Input: part model. Units: mm. Frame: model coordinates. Face numbers are marked on the shaded views. Coordinates: 2 decimals unless noted, no trailing zeros. Loops run counter-clockwise (first coordinate to the right, second up) from the corner with the lowest first, then second, coordinate; pieces in that order, holes last.
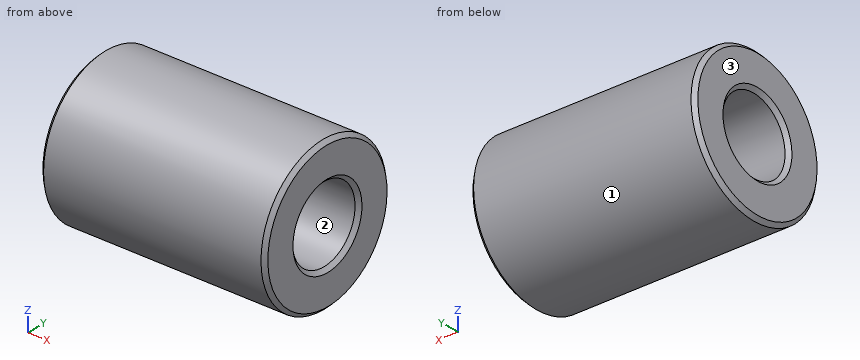
```python
from build123d import *

# Parameters (mm, degrees)
CHAMFER1_SIZE = 0.2


with BuildPart() as part:
    # Sketch1 → Revolve1 (revolve)
    with BuildSketch(Plane.XY, mode=Mode.PRIVATE) as revolve1_sk:
        Polygon((0, 3.7), (0, 2), (12, 2), (12, 3.7), (12, 4), (11.7, 4), (0.3, 4), (0, 4), align=None)
    revolve(revolve1_sk.sketch.rotate(Axis((12, 0, 0), (-1, 0, 0)), 270), axis=Axis((12, 0, 0), (-1, 0, 0)))

    # Chamfer1
    chamfer1_edges = [part.edges().sort_by_distance(p)[0] for p in [
        (0, 0, -4),
        (12, 0, -4),
        (12, 0, -2),
        (0, 0, -2),
    ]]
    chamfer(chamfer1_edges, length=CHAMFER1_SIZE)


solid = part.part
```
Item 1: Section query A-A (z = 0). Output: boundary loops of the cut face in (x, y).
Result:
outline: (0, -3.8) - (0.2, -4) - (11.8, -4) - (12, -3.8) - (12, -2.2) - (11.8, -2) - (0.2, -2) - (0, -2.2) - close; (0, 2.2) - (0.2, 2) - (11.8, 2) - (12, 2.2) - (12, 3.8) - (11.8, 4) - (0.2, 4) - (0, 3.8) - close
Item 2: Line query: L1, parallel to Y at x = 7.5, z = 0; L2, parallel to Z at x = 5, y = -1; L3, parallel to Z at x = 3.75, y = 1.25. Output: solid intervals per line, ascending.
Result:
L1: y = -4 to -2, 2 to 4
L2: z = -3.87 to -1.73, 1.73 to 3.87
L3: z = -3.8 to -1.56, 1.56 to 3.8
Item 3: Section query C-C (x = 4.75). Output: boundary loops of the cut face in (y, z).
Result:
outline: circle Ø8 at (0, 0); hole circle Ø4 at (0, 0)
Item 4: Contact query for flat-ended pins moving along their axis: P1, Ø3.5, axis at y = 0, z = 0, coming from the +X side; P2, Ø3, axis at x = 2, y = 2, coming from the -Z side; P3, Ø1, axis at x = 9, y = -1, coming from the +Z side. Output: stop coordinate, or through.
Result:
P1: passes through
P2: stops at z = -3.97
P3: stops at z = 3.97
Item 5: Mould query, pull axis Y, two halves, no side actions, for the marked faces 1, 2 and 3. Classes: +Y half, -Y half, draft (parallel to the pull), parting line (faces both ways), or undercut.
Result:
face 1: parting line
face 2: undercut
face 3: draft
